Could you check a few things on this model? Use its own coordinates, in mm. Face numbers are marked on the shaded views. A direction names the side the tool comes from. Coordinates: 2 decimals unless noted, no trailing zeros. Loops run counter-clockwise (first coordinate to the right, second up) from the corner with the lowest first, then second, coordinate; pieces in that order, holes last. Notation, with made-up numbers: M 19,24.25 L 33,24.25 A26 cw 33,54.25 Z; hole C 33,58.5 d10. An arc over 180 degrees is marked long. Write each question's results on one line, items separated by ' | '.
```python
from build123d import *

# Parameters (mm, degrees)
CLAMP_BODY_DEPTH          = 40
CLAMP_BODY_DEPTH_BACK     = 2
CLAMP_SCREW_HOLE_SKETCH_R = 5
CLAMP_SCREW_HOLE_10_DEPTH = 111.617355236
PIVOT_ARM_SKETCH_R        = 14
PIVOT_ARM_AND_BOSS_DEPTH  = 42
ARM_RIB_REACH             = 171.802
ARM_RIB_SKETCH_WALLS_W    = 433.168174749
ARM_RIB_SKETCH_WALLS_H    = 12
CLAMP_RIB_REACH           = 161.912
CLAMP_RIB_SKETCH_WALLS_W  = 402.175841481
CLAMP_RIB_SKETCH_WALLS_H  = 12
BORE_START                = -60
BORE_SKETCH_R             = 32
BORE_64_DEPTH             = 60


with BuildPart() as part:
    # Clamp Body Sketch → Clamp Body (new, two sides: drawn at the far end of the back side and taken through both)
    with BuildSketch(Plane.XY.offset(-CLAMP_BODY_DEPTH_BACK)):
        with BuildLine():
            ThreePointArc((30, -37.46998799), (17.305444592, -44.771883895), (3, -47.906158268))
            Line((3, -47.906158268), (3, -53.969677407))
            Line((3, -53.969677407), (3, -67.46998799))
            Line((3, -67.46998799), (30, -67.46998799))
            Line((30, -67.46998799), (30, -37.46998799))
        make_face()
        with BuildLine():
            ThreePointArc((3, -47.906158268), (0, 48), (-3, -47.906158268))
            Line((-3, -47.906158268), (-3, -31.859064644))
            ThreePointArc((-3, -31.859064644), (0, 32), (3, -31.859064644))
            Line((3, -31.859064644), (3, -47.906158268))
        make_face()
        with BuildLine():
            ThreePointArc((-3, -47.906158268), (-17.305444592, -44.771883895), (-30, -37.46998799))
            Line((-30, -37.46998799), (-30, -67.46998799))
            Line((-30, -67.46998799), (-3, -67.46998799))
            Line((-3, -67.46998799), (-3, -47.906158268))
        make_face()
    extrude(amount=CLAMP_BODY_DEPTH + CLAMP_BODY_DEPTH_BACK)

    # Clamp Screw Hole Sketch → Clamp Screw Hole _10 (cut, through all)
    with BuildSketch(Plane.ZY.offset(30)):
        with Locations((20, -52.46998799)):
            Circle(CLAMP_SCREW_HOLE_SKETCH_R)
    extrude(amount=-CLAMP_SCREW_HOLE_10_DEPTH, mode=Mode.SUBTRACT)

    # Pivot Arm Sketch → Pivot Arm and Boss (add)
    with BuildSketch(Plane.XY.offset(40)):
        with BuildLine():
            Line((40.319786094, 6), (40.319786094, -6))
            Line((40.319786094, -6), (84.701778719, -6))
            ThreePointArc((84.701778719, -6), (136, 0), (84.701778719, 6))
            Line((84.701778719, 6), (40.319786094, 6))
        make_face()
        with Locations((110, 0)):
            Circle(PIVOT_ARM_SKETCH_R, mode=Mode.SUBTRACT)
    extrude(amount=-PIVOT_ARM_AND_BOSS_DEPTH)

    # Arm Rib Sketch walls → Arm Rib (add, up to next)
    with BuildSketch(Plane(origin=(0, 26, 0), x_dir=(1, 0, 0), z_dir=(0, 1, 0)), mode=Mode.PRIVATE) as arm_rib_sk1:
        with Locations((64.5685648, -19)):
            Rectangle(ARM_RIB_SKETCH_WALLS_W, ARM_RIB_SKETCH_WALLS_H)
    arm_rib_tool1 = extrude(arm_rib_sk1.sketch, amount=-ARM_RIB_REACH, mode=Mode.PRIVATE) - part.part
    add(arm_rib_tool1.solids().sort_by_distance((64.568564799, 26, 19))[0])

    # Clamp Rib Sketch walls → Clamp Rib (add, up to next)
    with BuildSketch(Plane(origin=(0, -26, 0), x_dir=(1, 0, 0), z_dir=(0, 1, 0)), mode=Mode.PRIVATE) as clamp_rib_sk1:
        with Locations((70.17544468, -19)):
            Rectangle(CLAMP_RIB_SKETCH_WALLS_W, CLAMP_RIB_SKETCH_WALLS_H)
    clamp_rib_tool1 = extrude(clamp_rib_sk1.sketch, amount=CLAMP_RIB_REACH, mode=Mode.PRIVATE) - part.part
    add(clamp_rib_tool1.solids().sort_by_distance((70.17544468, -26, 19))[0])

    # Bore Sketch → Bore _64 (cut)
    with BuildSketch(Plane.XY.offset(40).offset(BORE_START)):
        Circle(BORE_SKETCH_R)
    extrude(amount=BORE_64_DEPTH, mode=Mode.SUBTRACT)


solid = part.part
```
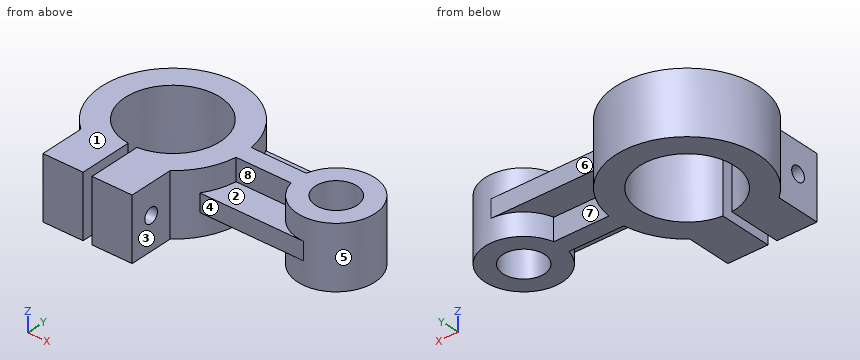
(1) Please list where these lines run through material, in increasing order: probe 1 along X at (y, z) = (16, 26.5); probe 2 along X at (y, z) = (-11.5, 7.5); probe 3 along X at (y, z) = (-19.5, 27). Write a range as from..to.
Reported:
probe 1: x = -45.25..-27.71, 27.71..45.25, 89.51..130.49 | probe 2: x = -46.6..-29.86, 29.86..46.6, 86.68..102.02, 117.98..133.32 | probe 3: x = -43.86..-25.37, 25.37..43.86, 92.8..127.2
(2) Which directions (+Z, -Z, +X, -X, +Y, -Y) give clear straight access to the entire face, cutting with the end or side of a thin tool? Please do the marked faces 4, 5, 6, 7 and 8.
Reported:
face 4: +Z, -Z, +X, -Y | face 5: none | face 6: +Z, -Z, +X, +Y | face 7: -Z, +Y | face 8: +Z, -Y
(3) Imagine slicing it at D-D, the plane x = -11.5. List the corners of the cut face in (y, z) for me, and give its area (3 significant figures).
Reported:
outline: M -67.47,-2 L -29.86,-2 L -29.86,40 L -67.47,40 Z; M 29.86,-2 L 46.6,-2 L 46.6,40 L 29.86,40 Z; hole C -52.47,20 d10 | area: 2,200 mm2
(4) Imagine slicing it at C-C, the plane x = 60. List the corners of the cut face in (y, z) for me.
Reported:
outline: M -26,13 L -6,13 L -6,-2 L 6,-2 L 6,13 L 26,13 L 26,25 L 6,25 L 6,40 L -6,40 L -6,25 L -26,25 Z
(5) Imagine slicing it at B-B, the plane y = 0. List the corners of the cut face in (x, z) for me, and give its area (3 significant figures).
Reported:
outline: M -48,-2 L -32,-2 L -32,40 L -48,40 Z; M 32,-2 L 96,-2 L 96,40 L 32,40 Z; M 124,-2 L 136,-2 L 136,40 L 124,40 Z | area: 3,860 mm2
(6) If we mould it in two halves opening along X, with no side actions, what happens to the marked faces 1, 2 and 3? For each: released by +X, released by -X, zero draft, split by the parting line, or undercut.
Reported:
face 1: zero draft | face 2: undercut | face 3: released by +X
(7) Will these pins go through, and if not, where does the flat tip stop? P1, Ø6, axis at x = 95.5, z = 21, coming from the +Y side; P2, Ø10.5, axis at y = -48.5, z = 19.5, coming from the -X side; P3, Ø10, axis at y = 5.5, z = 7.5, coming from the -X side.
Reported:
P1: stops at y = 26 | P2: stops at x = -30 | P3: stops at x = -48
(8) Imagine slicing it at A-A, the plane z = 20. List the corners of the cut face in (x, y) for me.
Reported:
outline: M -30,-67.47 L -3,-67.47 L -3,-57.47 L -30,-57.47 Z; M -30,-47.47 L -3,-47.47 L -3,-31.86 A32 cw long 3,-31.86 L 3,-47.47 L 30,-47.47 L 30,-37.47 A48 ccw 40.35,-26 L 110,-26 A26 ccw 110,26 L 40.35,26 A48 ccw long -30,-37.47 Z; M 3,-67.47 L 30,-67.47 L 30,-57.47 L 3,-57.47 Z; hole C 110,0 d28
